```python
from build123d import *

# Parameters (mm, degrees)
EXTRUDE_1_DEPTH = 30


with BuildPart() as part:
    # 草图1 → 凸台-拉伸1 (new body)
    with BuildSketch(Plane.XY):
        Polygon((0, 0), (0, 670), (50, 670), (210, 50), (210, 0), align=None)
    extrude(amount=EXTRUDE_1_DEPTH)


solid = part.part
```
Model file for the job. Use its own axes, mm. Round coordinates to 2 decimals unless told otherwise and drop trailing zeros. Loops run counter-clockwise (first coordinate to the right, second up) from the corner with the lowest first, then second, coordinate; pieces in that order, holes last. Notation, with made-up numbers: M 32.25,0.25 L 77.25,0.25 A17 ccw 77.25,21.25 Z; hole C 54.5,30 d7. An arc over 180 degrees is marked long. Put each result on its own line as item: value. Start each with the question number.
Item 1: Cut at C-C (y = 262). List the corners of the cut face in (x, z).
Item 2: Drill centre lines: line 1 along X through (y, z) = (132, 3.5); line 2 along X through (y, z) = (467.5, 23.5). Where is each one in solid material? Low to high.
Item 3: Cut at A-A (z = 7.75). List the corners of the cut face in (x, y), then the cut area to 3 significant figures.
Item 4: Cut at B-B (x = 182). List the corners of the cut face in (y, z), then the cut area to 4 significant figures.
Answer block:
1. outline: M 0,0 L 155.29,0 L 155.29,30 L 0,30 Z
2. line 1: 0 to 188.84
2. line 2: 0 to 102.26
3. outline: M 0,0 L 210,0 L 210,50 L 50,670 L 0,670 Z
3. area: 91,100 mm2
4. outline: M 0,0 L 158.5,0 L 158.5,30 L 0,30 Z
4. area: 4,755 mm2
